```python
from build123d import *

# Parameters (mm, degrees)
BRACKET_BODY_DEPTH        = 46
TAPERED_SIDE_CUT_DEPTH    = 46
BORE_SKETCH_R             = 7
THROUGH_BORE_14_DEPTH     = 46
BORE_EDGE_FILLET_R0_5_A_R = 0.5
BORE_EDGE_FILLET_R0_5_B_R = 0.5
STEP_EDGE_FILLET_R0_5_R   = 0.5


with BuildPart() as part:
    # Bracket Profile Sketch → Bracket Body (new body)
    with BuildSketch(Plane.XY):
        Polygon((0, 0), (22, 0), (22, 12), (12, 12), (12, 55), (-10, 55), (-10, 43), (0, 43), align=None)
    extrude(amount=BRACKET_BODY_DEPTH)

    # Taper Cut Sketch → Tapered Side Cut (cut)
    with BuildSketch(Plane(origin=(22, 0, 0), x_dir=(0, 0, -1), z_dir=(1, 0, 0))):
        Polygon((-46, 0), (-35, 55), (-46, 55), align=None)
        Polygon((0, 0), (0, 55), (-11, 55), align=None)
    extrude(amount=-TAPERED_SIDE_CUT_DEPTH, mode=Mode.SUBTRACT)

    # Bore Sketch → Through Bore Ø14 (cut)
    with BuildSketch(Plane.ZY):
        with Locations(Location((23, 27.5, 0), (0, 0, 270))):
            Circle(BORE_SKETCH_R)
    extrude(amount=-THROUGH_BORE_14_DEPTH, mode=Mode.SUBTRACT)

    # Bore Edge Fillet R0.5 A
    bore_edge_fillet_r0_5_a_edges = [part.edges().sort_by_distance(p)[0] for p in [
        (12, 34.5, 23),
    ]]
    fillet(bore_edge_fillet_r0_5_a_edges, radius=BORE_EDGE_FILLET_R0_5_A_R)

    # Bore Edge Fillet R0.5 B
    bore_edge_fillet_r0_5_b_edges = [part.edges().sort_by_distance(p)[0] for p in [
        (0, 34.5, 23),
    ]]
    fillet(bore_edge_fillet_r0_5_b_edges, radius=BORE_EDGE_FILLET_R0_5_B_R)

    # Step Edge Fillet R0.5
    step_edge_fillet_r0_5_edges = [part.edges().sort_by_distance(p)[0] for p in [
        (12, 12, 23),
    ]]
    fillet(step_edge_fillet_r0_5_edges, radius=STEP_EDGE_FILLET_R0_5_R)


solid = part.part
```
CAD build for the part. Positions are in the model's coordinates, mm. A direction names the side the tool comes from. Round coordinates to 2 decimals unless told otherwise and drop trailing zeros. Order: outer loops, then holes, each group sorted by start corner. A loop starts at its lowest first (then second) coordinate and runs counter-clockwise, first axis right, second up.
Item 1: Probe line 1 along X through (y, z) = (22, 15.5); line 2 along Y through (x, z) = (5, 28.5). List the from-to ranges inside material, lowest first.
Item 2: Pin check, flat tips, straight feed: pin 1 (5 mm diameter, centred on x = 15.5, z = 20, fed in from +Y); pin 2 (10 mm diameter, centred on x = 13.5, y = 17.5, fed in from -Z); pin 3 (6 mm diameter, centred on y = 35, z = 24, fed in from +X); pin 4 (1 mm diameter, centred on x = 13, y = 44, fed in from -Z) (3 decimals). Stop position of each tip, or through.
Item 3: Tool access for faces 1 (the face through (-5, 43, 23)), 2 (the face through (6.224, 27.115, 40.577)): list every direction of +Z, -Z, +X, -X, +Y, -Y with a clear straight run to the whole face (end or side of a thin tool).
Item 4: Saw through at D-D on z = 34. Write the cut outline in (x, y).
Item 5: Saw through at A-A on z = 23. Write the cut outline in (x, y).
Item 6: Mould opens along Y. For faces 3 (the face through (17, 12, 23)), 4 (the face through (12, 33.5, 18.2)), 5 (the face through (5.923, 21.034, 20.319)) say: pulls with the +Y half, pulls with the -Y half, needs draft (parallel to the pull), parting line crosses it, or undercut.
Item 7: Saw through at B-B on y = 27.5. Write the cut outline in (x, z).
Item 8: Saw through at C-C on x = 10.5. Write the cut outline in (y, z).
Reported:
1. line 1: x = 0 to 12
1. line 2: y = 0 to 23.17, 31.83 to 55
2. pin 1: stops at y = 12
2. pin 2: stops at z = 2.55
2. pin 3: stops at x = 12
2. pin 4: passes through
3. face 1: +Z, -Z, -X, -Y
3. face 2: +Z, +X, -X, +Y
4. outline: (-10, 43) - (0, 43) - (0, 0) - (22, 0) - (22, 12) - (12.5, 12) arc R0.5 cw to (12, 12.5) - (12, 55) - (-10, 55) - close
5. outline: (-10, 43) - (0, 43) - (0, 35) arc R0.5 ccw to (0.5, 34.5) - (11.5, 34.5) arc R0.5 ccw to (12, 35) - (12, 55) - (-10, 55) - close; (0, 0) - (22, 0) - (22, 12) - (12.5, 12) arc R0.5 cw to (12, 12.5) - (12, 20) arc R0.5 ccw to (11.5, 20.5) - (0.5, 20.5) arc R0.5 ccw to (0, 20) - close
6. face 3: pulls with the +Y half
6. face 4: needs draft
6. face 5: undercut
7. outline: (0, 5.5) - (12, 5.5) - (12, 15.5) arc R0.5 ccw to (11.5, 16) - (0.5, 16) arc R0.5 ccw to (0, 15.5) - close; (0, 30.5) arc R0.5 ccw to (0.5, 30) - (11.5, 30) arc R0.5 ccw to (12, 30.5) - (12, 40.5) - (0, 40.5) - close
8. outline: (0, 0) - (55, 11) - (55, 35) - (0, 46) - close; hole circle Ø14 at (27.5, 23)
